```python
from build123d import *

# Parameters (mm, degrees)
SKETCH_1_W                  = 55
SKETCH_1_H                  = 60
EXTRUDE_1_DEPTH             = 5
HOLE_WIZARD_M4_1_AT_2_COUNT = 2
HOLE_WIZARD_M4_1_AT_2_PITCH = 36


with BuildPart() as part:
    # 草图1 → 凸台-拉伸1 (new, symmetric)
    with BuildSketch(Plane.XY):
        Rectangle(SKETCH_1_W, SKETCH_1_H)
    extrude(amount=EXTRUDE_1_DEPTH, both=True)

    # 草图4 → M4 螺纹孔1 (revolve, cut)
    with BuildSketch(Plane(origin=(18, -30, 0), x_dir=(0, 0, -1), z_dir=(1, 0, 0))):
        Polygon((0, 0), (0, 12.491420021), (1.65, 11.5), (1.65, 0), align=None)
    hole_wizard_m4_1 = revolve(axis=Axis((18, -36.35, 0), (0, 1, 0)), mode=Mode.SUBTRACT)

    # M4 螺纹孔1 at 2: M4 螺纹孔1 ×2
    with Locations(*[(-i * HOLE_WIZARD_M4_1_AT_2_PITCH, 0, 0) for i in range(1, HOLE_WIZARD_M4_1_AT_2_COUNT)]):
        add(hole_wizard_m4_1, mode=Mode.SUBTRACT)

    # 镜向1: M4 螺纹孔1 across plane
    add(hole_wizard_m4_1.mirror(Plane.ZX), mode=Mode.SUBTRACT)

    # 镜向1 copy 1 sketch → 镜向1 copy 1 (revolve, cut)
    with BuildSketch(Plane(origin=(-18, 30, 0), x_dir=(0, 0, -1), z_dir=(1, 0, 0))):
        Polygon((0, 0), (0, -12.491420021), (1.65, -11.5), (1.65, 0), align=None)
    revolve(axis=Axis((-18, 36.35, 0), (0, 1, 0)), mode=Mode.SUBTRACT)


solid = part.part
```
CAD build for the part. Positions are in the model's coordinates, mm. A direction names the side the tool comes from. Give positions to 0.01 mm unless a question says otherwise; leave off trailing zeros. Loops run counter-clockwise (first coordinate to the right, second up) from the corner with the lowest first, then second, coordinate; pieces in that order, holes last. Notation, with made-up numbers: (87, 20.25) - (98, 20.25) arc R6 cw to (98, 24.25) - close; hole circle Ø1 at (-8.75, 42). An arc over 180 degrees is marked (long way). Put each result on its own line as item: value.
Q1. Mould opens along Z. For faces 1 (the face through (-19.636, -24.33, 0.215)), 2 (the face through (0, 0, 5)), 3 (the face through (0, 30, 0)) say: pulls with the +Z half, pulls with the -Z half, needs draft (parallel to the pull), parting line crosses it, or undercut.
Filled in:
face 1: undercut
face 2: pulls with the +Z half
face 3: needs draft
Q2. Flat gauge pins, fed straight in: pin 1 (2 mm diameter, centred on x = -18, z = 0, fed in from -Y); pin 2 (2 mm diameter, centred on x = -18, z = 0, fed in from +Y); pin 3 (3 mm diameter, centred on x = 18, z = 0, fed in from -Y). Where does each tip first touch, or does it go through?
Filled in:
pin 1: stops at y = -18.11
pin 2: stops at y = 18.11
pin 3: stops at y = -18.41
Q3. Probe line 1 along X through (y, z) = (-27.5, 0); line 2 along Z through (x, y) = (-18, 22.75); line 3 along X through (y, z) = (-23, 0.75). List the from-to ranges inside material, lowest first.
Filled in:
line 1: x = -27.5 to -19.65, -16.35 to 16.35, 19.65 to 27.5
line 2: z = -5 to -1.65, 1.65 to 5
line 3: x = -27.5 to -19.47, -16.53 to 16.53, 19.47 to 27.5
Q4. Slice it at A-A (y = -23.5). Give the cut face in (x, z), plus the area to 3 significant figures.
Filled in:
outline: (-27.5, -5) - (27.5, -5) - (27.5, 5) - (-27.5, 5) - close; hole circle Ø3.3 at (-18, 0); hole circle Ø3.3 at (18, 0)
area: 533 mm²
Q5. Tool access for faces 4 (the face through (16.364, -24.33, 0.215)), 5 (the face through (0, 0, -5)), 6 (the face through (16.364, 24.33, 0.215)): list every direction of +Z, -Z, +X, -X, +Y, -Y with a clear straight run to the whole face (end or side of a thin tool).
Filled in:
face 4: -Y
face 5: -Z, +X, -X, +Y, -Y
face 6: +Y
